The model under review builds one solid part; all positions refer to its coordinate system, in mm. Give positions to 0.01 mm unless a question says otherwise; leave off trailing zeros. Loops run counter-clockwise (first coordinate to the right, second up) from the corner with the lowest first, then second, coordinate; pieces in that order, holes last. Notation, with made-up numbers: M 12.25,19.5 L 46.25,19.5 A20 ccw 46.25,36.5 Z; hole C -14.5,-2 d11. An arc over 180 degrees is marked long. One line per item, written item: value. Start each with the question number.
Q1. We need section A-A on y = 17.5. Write out the cut boundary in (x, z), plus the area to 3 significant figures.
Q2. We need section B-B on x = 50. Write out the cut boundary in (y, z).
Q3. We need section D-D on y = 0. Write out the cut boundary in (x, z), plus the area to 3 significant figures.
Q4. We need section C-C on z = -0.6. Write out the cut boundary in (x, y).
Q5. To check wall thickness, follow line 1 along X through (y, z) = (-2, -0.2); line 2 along Y through (x, z) = (-25, -0.35); line 3 along X through (y, z) = (3, 0.8). State the ranges of each line that lie inside material, in increasing order. Write a range as from..to.
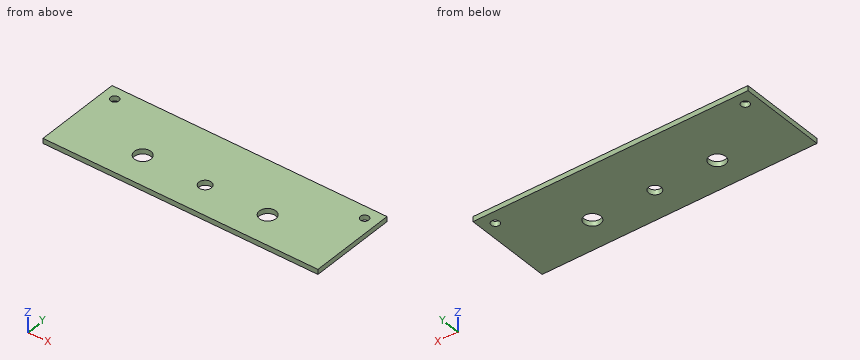
```python
from build123d import *

# Parameters (mm, degrees)
SKETCH_1_W          = 110
SKETCH_1_H          = 25
SKETCH_1_R          = 3.3
EXTRUDE_1_DEPTH     = 1
SKETCH_2_R          = 2.5
CUT_EXTRUDE_1_DEPTH = 10
SKETCH_3_W          = 110
SKETCH_3_H          = 2
EXTRUDE_2_DEPTH     = 10
SKETCH_4_R          = 1.65
CUT_EXTRUDE_2_DEPTH = 10


with BuildPart() as part:
    # 草图1 → 凸台-拉伸1 (new, symmetric)
    with BuildSketch(Plane.XY):
        Rectangle(SKETCH_1_W, SKETCH_1_H)
        with Locations((-25, 0)):
            Circle(SKETCH_1_R, mode=Mode.SUBTRACT)
        with Locations((25, 0)):
            Circle(SKETCH_1_R, mode=Mode.SUBTRACT)
    extrude(amount=EXTRUDE_1_DEPTH, both=True)

    # 草图2 → 切除-拉伸1 (cut)
    with BuildSketch(Plane.XY.offset(1)):
        Circle(SKETCH_2_R)
    extrude(amount=-CUT_EXTRUDE_1_DEPTH, mode=Mode.SUBTRACT)

    # 草图3 → 凸台-拉伸2 (add)
    with BuildSketch(Plane(origin=(0, 12.5, 0), x_dir=(1, 0, 0), z_dir=(0, 1, 0))):
        Rectangle(SKETCH_3_W, SKETCH_3_H)
    extrude(amount=EXTRUDE_2_DEPTH)

    # 草图4 → 切除-拉伸2 (cut)
    with BuildSketch(Plane(origin=(0, 0, -1), x_dir=(-1, 0, 0), z_dir=(0, 0, -1))):
        with Locations((-50, 17.5)):
            Circle(SKETCH_4_R)
        with Locations((50, 17.5)):
            Circle(SKETCH_4_R)
    extrude(amount=-CUT_EXTRUDE_2_DEPTH, mode=Mode.SUBTRACT)


solid = part.part
```
Solved:
1. outline: M -55,-1 L -51.65,-1 L -51.65,1 L -55,1 Z; M -48.35,-1 L 48.35,-1 L 48.35,1 L -48.35,1 Z; M 51.65,-1 L 55,-1 L 55,1 L 51.65,1 Z
1. area: 207 mm2
2. outline: M -12.5,-1 L 15.85,-1 L 15.85,1 L -12.5,1 Z; M 19.15,-1 L 22.5,-1 L 22.5,1 L 19.15,1 Z
3. outline: M -55,-1 L -28.3,-1 L -28.3,1 L -55,1 Z; M -21.7,-1 L -2.5,-1 L -2.5,1 L -21.7,1 Z; M 2.5,-1 L 21.7,-1 L 21.7,1 L 2.5,1 Z; M 28.3,-1 L 55,-1 L 55,1 L 28.3,1 Z
3. area: 184 mm2
4. outline: M -55,-12.5 L 55,-12.5 L 55,22.5 L -55,22.5 Z; hole C -50,17.5 d3.3; hole C -25,0 d6.6; hole C 0,0 d5; hole C 25,0 d6.6; hole C 50,17.5 d3.3
5. line 1: -55..-27.62, -22.38..-1.5, 1.5..22.38, 27.62..55
5. line 2: -12.5..-3.3, 3.3..22.5
5. line 3: -55..-26.37, -23.63..23.63, 26.37..55
